from build123d import *

# Parameters (mm, degrees)
SKETCH_1_W          = 1000
SKETCH_1_H          = 80
EXTRUDE_1_DEPTH     = 50
SHELL_1_T           = -3
FILLET_1_R          = 5
SKETCH_3_R          = 17.6
CUT_EXTRUDE_2_DEPTH = 505.083326445
SKETCH_4_R          = 3.4
CUT_EXTRUDE_3_DEPTH = 10
SKETCH_5_R          = 2.5
CUT_EXTRUDE_4_DEPTH = 10
SKETCH_6_R          = 2.1
CUT_EXTRUDE_5_DEPTH = 10


with BuildPart() as part:
    # 草图1 → 凸台-拉伸1 (new body)
    with BuildSketch(Plane.XY):
        Rectangle(SKETCH_1_W, SKETCH_1_H)
    extrude(amount=EXTRUDE_1_DEPTH)

    # 抽壳1
    shell_1_openings = [part.faces().sort_by_distance(p)[0] for p in [
        (-500, 0, 25),
        (500, 0, 25),
    ]]
    offset(amount=SHELL_1_T, openings=shell_1_openings, kind=Kind.INTERSECTION)

    # 圆角1
    fillet_1_edges = [part.edges().sort_by_distance(p)[0] for p in [
        (0, -40, 50),
        (0, -40, 0),
        (0, 40, 0),
        (0, 40, 50),
    ]]
    fillet(fillet_1_edges, radius=FILLET_1_R)

    # 草图3 → 切除-拉伸2 (cut, through all)
    with BuildSketch(Plane(origin=(0, 0, 0), x_dir=(-1, 0, 0), z_dir=(0, 0, -1))):
        with Locations((-292, 0)):
            Circle(SKETCH_3_R)
        with Locations((292, 0)):
            Circle(SKETCH_3_R)
    extrude(amount=-CUT_EXTRUDE_2_DEPTH, mode=Mode.SUBTRACT)

    # 草图4 → 切除-拉伸3 (cut)
    with BuildSketch(Plane(origin=(0, 0, 0), x_dir=(-1, 0, 0), z_dir=(0, 0, -1))):
        with Locations((-329.5, 20)):
            Circle(SKETCH_4_R)
        with Locations((-329.5, -20)):
            Circle(SKETCH_4_R)
        with Locations((-254.5, 20)):
            Circle(SKETCH_4_R)
        with Locations((-254.5, -20)):
            Circle(SKETCH_4_R)
        with Locations((254.5, 20)):
            Circle(SKETCH_4_R)
        with Locations((254.5, -20)):
            Circle(SKETCH_4_R)
        with Locations((329.5, 20)):
            Circle(SKETCH_4_R)
        with Locations((329.5, -20)):
            Circle(SKETCH_4_R)
    extrude(amount=-CUT_EXTRUDE_3_DEPTH, mode=Mode.SUBTRACT)

    # 草图5 → 切除-拉伸4 (cut)
    with BuildSketch(Plane(origin=(0, 0, 0), x_dir=(-1, 0, 0), z_dir=(0, 0, -1))):
        Circle(SKETCH_5_R)
        with Locations((25, 0)):
            Circle(SKETCH_5_R)
    extrude(amount=-CUT_EXTRUDE_4_DEPTH, mode=Mode.SUBTRACT)

    # 草图6 → 切除-拉伸5 (cut)
    with BuildSketch(Plane.XZ.offset(40)):
        with Locations(Location((110.1, 21.5, 0), (0, 0, 270))):
            Circle(SKETCH_6_R)
        with Locations(Location((-250.1, 21.5, 0), (0, 0, 270))):
            Circle(SKETCH_6_R)
    extrude(amount=-CUT_EXTRUDE_5_DEPTH, mode=Mode.SUBTRACT)


solid = part.part
Check sheet for the modelled part. Datum: model origin and axes. Units: mm. A direction names the side the tool comes from. Coordinates: 2 decimals unless noted, no trailing zeros. Loops run counter-clockwise (first coordinate to the right, second up) from the corner with the lowest first, then second, coordinate; pieces in that order, holes last. Notation, with made-up numbers: (33, -33.5) -> (50, -33.5) arc R25 cw to (50, 5.5) -> close; hole circle Ø6 at (-11, 86.5). An arc over 180 degrees is marked (long way). Write item = value, one per line. Start each with the question number.
1. Draft check along X on faces 3 (the cylindrical face through (309.583, 0.774, 1.479)), 4 (the flat face through (-7, -37, 25)), 5 (the flat face through (-500, -0.2, 2.7)), 6 (the flat face through (500, -0.2, 2.7)). Enter one of: released by +X, released by -X, zero draft, split by the parting line, or undercut.
2. Depth check by flat-ended pin: P1, Ø6, axis at x = 329.5, y = -20, coming from the -Z side. Enter the tip coordinate at first touch or a pass-through.
3. Tool access check on faces 1 (the flat face through (-7, 40, 25)), 2 (the flat face through (-7, 1, 3)). Record the directions out of +Z, -Z, +X, -X, +Y, -Y that give a thin tool (end or side, any length) a straight path to the whole face; none if there is none.
4. Section check A-A on x = 145. Record the cut outline in (y, z).
5. Material ranges on line 1 (Z direction, x = 199, y = -12.5); line 2 (Y direction, x = -425.5, z = 29); line 3 (Y direction, x = 329.5, z = 1.85), recorded low to high.
Responses:
q1.face_3 = undercut
q1.face_4 = zero draft
q1.face_5 = released by -X
q1.face_6 = released by +X
q2.P1 = 47
q3.face_1 = +Z, -Z, +X, -X, +Y
q3.face_2 = +X, -X
q4.outline = (-40, 5) arc R5 ccw to (-35, 0) -> (35, 0) arc R5 ccw to (40, 5) -> (40, 45) arc R5 ccw to (35, 50) -> (-35, 50) arc R5 ccw to (-40, 45) -> close; hole (-37, 3) -> (37, 3) -> (37, 47) -> (-37, 47) -> close
q5.line_1 = 0 to 3, 47 to 50
q5.line_2 = -40 to -37, 37 to 40
q5.line_3 = -38.88 to -23.4, -16.6 to 16.6, 23.4 to 38.88
